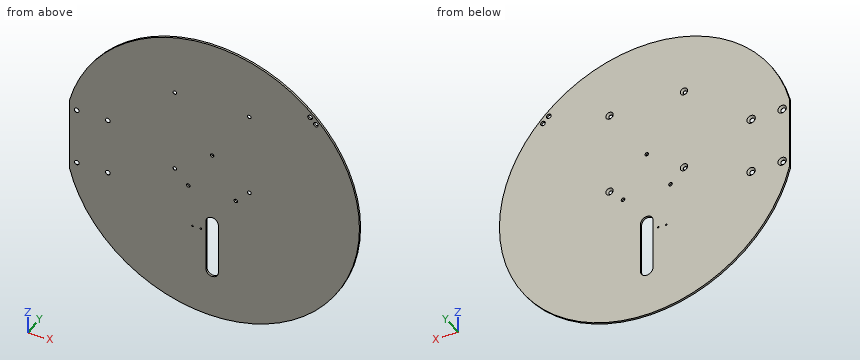
```python
from build123d import *

# Parameters (mm, degrees)
SKETCH1_R             = 142.5
BOSS_EXTRUDE1_DEPTH   = 2
SKETCH3_R             = 1.75
CUT_EXTRUDE1_DEPTH    = 10
CIRPATTERN1_COUNT     = 3
SKETCH5_R             = 2.25
CUT_EXTRUDE2_DEPTH    = 10
CUT_EXTRUDE3_DEPTH    = 202.5353567
SKETCH7_R             = 1.75
CUT_EXTRUDE4_DEPTH    = 10
CHAMFER1_SIZE         = 1.8
CHAMFER2_SIZE         = 1.8
M2_TAPPED_HOLE1_D     = 1.6
M2_TAPPED_HOLE1_DEPTH = 5.2
M2_TAPPED_HOLE1_TIP   = 0.480688495
SKETCH9_W             = 15.607073654
SKETCH9_H             = 79.285494628
CUT_EXTRUDE5_DEPTH    = 10


with BuildPart() as part:
    # Sketch1 → Boss-Extrude1 (new body)
    with BuildSketch(Plane(origin=(0, 0, 0), x_dir=(1, 0, 0), z_dir=(0, 1, 0))):
        with Locations(Location((0, 0, 0), (0, 0, 270))):
            Circle(SKETCH1_R)
    extrude(amount=BOSS_EXTRUDE1_DEPTH)

    # Sketch3 → Cut-Extrude1 (cut)
    with BuildSketch(Plane(origin=(0, 2, 0), x_dir=(1, 0, 0), z_dir=(0, 1, 0))):
        with Locations(Location((0, -26.5, 0), (0, 0, 270))):
            Circle(SKETCH3_R)
    cut_extrude1 = extrude(amount=-CUT_EXTRUDE1_DEPTH, mode=Mode.SUBTRACT)

    # CirPattern1: Cut-Extrude1 ×3 about axis
    cirpattern1_axis = Axis((0, 0, 0), (0, 1, 0))
    for i in range(1, CIRPATTERN1_COUNT):
        add(cut_extrude1.rotate(cirpattern1_axis, i * 360 / CIRPATTERN1_COUNT), mode=Mode.SUBTRACT)

    # Sketch5 → Cut-Extrude2 (cut)
    with BuildSketch(Plane(origin=(0, 2, 0), x_dir=(1, 0, 0), z_dir=(0, 1, 0))):
        with Locations(Location((94.711308368, -100.368162618, 0), (0, 0, 270))):
            Circle(SKETCH5_R)
        with Locations(Location((100.368162618, -94.711308368, 0), (0, 0, 270))):
            Circle(SKETCH5_R)
        with Locations(Location((-130.892369907, 27.5, 0), (0, 0, 270))):
            Circle(SKETCH5_R)
        with Locations(Location((-130.892369907, -27.5, 0), (0, 0, 270))):
            Circle(SKETCH5_R)
        with Locations(Location((-100.892369907, -27.5, 0), (0, 0, 270))):
            Circle(SKETCH5_R)
        with Locations(Location((-100.892369907, 27.5, 0), (0, 0, 270))):
            Circle(SKETCH5_R)
    extrude(amount=-CUT_EXTRUDE2_DEPTH, mode=Mode.SUBTRACT)

    # Sketch6 → Cut-Extrude3 (cut, through all)
    with BuildSketch(Plane(origin=(0, 2, 0), x_dir=(1, 0, 0), z_dir=(0, 1, 0))):
        with BuildLine():
            Line((-6, 45), (-6, 95))
            ThreePointArc((-6, 95), (0, 101), (6, 95))
            Line((6, 95), (6, 45))
            ThreePointArc((6, 45), (0, 39), (-6, 45))
        make_face()
    extrude(amount=-CUT_EXTRUDE3_DEPTH, mode=Mode.SUBTRACT)

    # Sketch7 → Cut-Extrude4 (cut)
    with BuildSketch(Plane.XZ):
        with Locations(Location((36, 0, 0), (0, 0, 270))):
            Circle(SKETCH7_R)
        with Locations(Location((-36, 0, 0), (0, 0, 270))):
            Circle(SKETCH7_R)
        with Locations(Location((-36, 80, 0), (0, 0, 270))):
            Circle(SKETCH7_R)
        with Locations(Location((36, 80, 0), (0, 0, 270))):
            Circle(SKETCH7_R)
    extrude(amount=-CUT_EXTRUDE4_DEPTH, mode=Mode.SUBTRACT)

    # Chamfer1
    chamfer1_edges = [part.edges().sort_by_distance(p)[0] for p in [
        (36, 2, 1.75),
        (-36, 2, 1.75),
        (-36, 2, 81.75),
        (36, 2, 81.75),
    ]]
    chamfer(chamfer1_edges, length=CHAMFER1_SIZE)

    # Chamfer2
    chamfer2_edges = [part.edges().sort_by_distance(p)[0] for p in [
        (-130.892369907, 2, -29.75),
        (-130.892369907, 2, 25.25),
        (-100.892369907, 2, 25.25),
        (-100.892369907, 2, -29.75),
    ]]
    chamfer(chamfer2_edges, length=CHAMFER2_SIZE)

    # M2 Tapped Hole1
    with Locations(Plane(origin=(-10.95, 0, -54.5), x_dir=(0, 0, -1), z_dir=(0, -1, 0))):
        with Locations((0, 0), (0, -8)):
            Hole(M2_TAPPED_HOLE1_D / 2, depth=M2_TAPPED_HOLE1_DEPTH)
            with Locations((0, 0, -(M2_TAPPED_HOLE1_DEPTH + M2_TAPPED_HOLE1_TIP / 2))):  # 118° drill point
                Cone(0, M2_TAPPED_HOLE1_D / 2, M2_TAPPED_HOLE1_TIP, mode=Mode.SUBTRACT)

    # Sketch9 → Cut-Extrude5 (cut)
    with BuildSketch(Plane(origin=(0, 2, 0), x_dir=(1, 0, 0), z_dir=(0, 1, 0))):
        with Locations((-145.803536827, 0)):
            Rectangle(SKETCH9_W, SKETCH9_H)
    extrude(amount=-CUT_EXTRUDE5_DEPTH, mode=Mode.SUBTRACT)


solid = part.part
```
Input: part model. Units: mm. Frame: model coordinates. Coordinates: 2 decimals unless noted, no trailing zeros. Write each loop counter-clockwise with the first axis right and the second up, starting at its lowest first coordinate (ties: lowest second). Pieces come first, ordered by that corner, then holes. Notation, with made-up numbers: (82.25, 52) - (128.25, 52) arc R21 cw to (128.25, 89) - close; hole circle Ø4 at (60, 7). An arc over 180 degrees is marked (long way). Put each result on its own line as item: value. Start each with the question number.
1) Cut plane D-D (z = 50). Return the cut outline in (x, y), plus the area to 3 significant figures.
2) Contact query for flat-ended pins moving along their axis: pin 1 (1 mm diameter, centred on y = 1.5, z = -72.5, fed in from -X); pin 2 (1 mm diameter, centred on x = -25.5, y = 0.5, fed in from +Z); pin 3 (1 mm diameter, centred on y = 1.5, z = -33, fed in from +X). Output: stop coordinate, or through.
3) Cut plane A-A (y = 0.6). State how many separate pieces and enclosed holes the cut face has, plus the area to 3 significant figures.
4) Cut plane B-B (z = -91.5). Return the cut outline in (x, y).
5) Ray query, L1, parallel to X at y = 0.1, z = 0; L2, parallel to X at y = 0.1, z = 27.5; L3, parallel to X at y = 0.6, z = -13.25. Return the intervals inside material, ascending.
6) Cut plane C-C (x = 56.5). Return the cut outline in (y, z), plus the area to 3 significant figures.
Resolved:
1. outline: (-133.44, 0) - (133.44, 0) - (133.44, 2) - (-133.44, 2) - close
1. area: 534 mm2
2. pin 1: stops at x = -122.97
2. pin 2: stops at z = 140.29
2. pin 3: stops at x = 138.74
3. separate pieces: 1
3. enclosed holes: 16
3. area: 62,700 mm2
4. outline: (-109.24, 0) - (-6, 0) - (-6, 2) - (-109.24, 2) - close; (6, 0) - (109.24, 0) - (109.24, 2) - (6, 2) - close
5. L1: x = -138 to -37.75, -34.25 to 34.25, 37.75 to 142.5
5. L2: x = -138 to -133.14, -128.64 to -103.14, -98.64 to -1.44, 1.44 to 139.82
5. L3: x = -138 to -24.7, -21.2 to 21.2, 24.7 to 141.88
6. outline: (0, -130.82) - (2, -130.82) - (2, 130.82) - (0, 130.82) - close
6. area: 523 mm2
